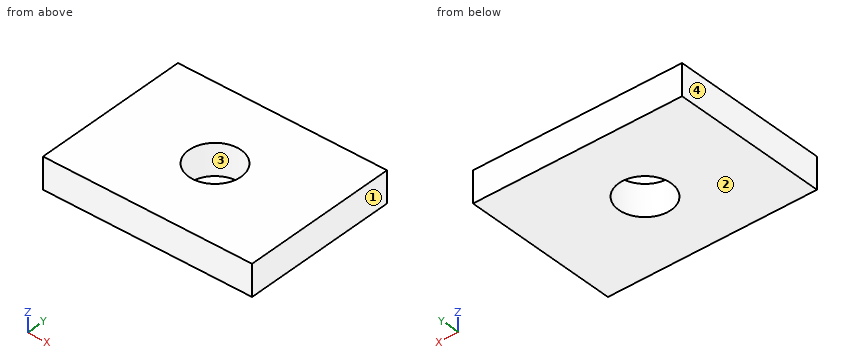
from build123d import *

# Parameters (mm, degrees)
SKETCH1_W           = 40
SKETCH1_H           = 30
BOSS_EXTRUDE1_DEPTH = 6
SKETCH2_R           = 5
CUT_EXTRUDE1_DEPTH  = 6


with BuildPart() as part:
    # Sketch1 → Boss-Extrude1 (new body)
    with BuildSketch(Plane.XY):
        with Locations((-26.669019685, -3.132226563)):
            Rectangle(SKETCH1_W, SKETCH1_H)
    extrude(amount=BOSS_EXTRUDE1_DEPTH)

    # Sketch2 → Cut-Extrude1 (cut)
    with BuildSketch(Plane.XY.offset(6)):
        with Locations((-26.669019685, -3.132226563)):
            Circle(SKETCH2_R)
    extrude(amount=-CUT_EXTRUDE1_DEPTH, mode=Mode.SUBTRACT)


solid = part.part
Here's how the part is built. I have some questions about the finished solid (model axes, mm). Face numbers are marked on the shaded views. Coordinates: 2 decimals unless noted, no trailing zeros. Order: outer loops, then holes, each group sorted by start corner. A loop starts at its lowest first (then second) coordinate and runs counter-clockwise, first axis right, second up. Notation, with made-up numbers: M 14.5,-31 L 44.5,-31 A23 cw 44.5,-13 Z; hole C 58.5,-6.5 d1. An arc over 180 degrees is marked long. Answer as CSV lines item,"result".
Item 1: Imagine slicing it at B-B on z = 2.1. Write out the boundary of the cut face in (x, y).
Results found:
outline,"M -46.67,-18.13 L -6.67,-18.13 L -6.67,11.87 L -46.67,11.87 Z; hole C -26.67,-3.13 d10"
Item 2: We'd pull the mould along X, two halves only. Please class the marked faces 1, 2, 3 and 4: +X half, -X half, draft (parallel to the pull), parting line (faces both ways), or undercut.
Results found:
face 1,"+X half"
face 2,"draft"
face 3,"undercut"
face 4,"-X half"
Item 3: Imagine slicing it at A-A on y = -7.25. Write out the boundary of the cut face in (x, z).
Results found:
outline,"M -46.67,0 L -29.51,0 L -29.51,6 L -46.67,6 Z; M -23.83,0 L -6.67,0 L -6.67,6 L -23.83,6 Z"
Item 4: If I drill on line 1 (X direction, y = -3, z = 3.1); line 2 (Y direction, x = -24, z = 5.45); line 3 (Y direction, x = -27, z = 3.7), over which ranges is the centre line in solid material (lowest first)?
Results found:
line 1,"-46.67 to -31.67, -21.67 to -6.67"
line 2,"-18.13 to -7.36, 1.1 to 11.87"
line 3,"-18.13 to -8.12, 1.86 to 11.87"
Item 5: Imagine slicing it at C-C on y = -4. Write out the boundary of the cut face in (x, z), plus the area to 3 significant figures.
Results found:
outline,"M -46.67,0 L -31.59,0 L -31.59,6 L -46.67,6 Z; M -21.74,0 L -6.67,0 L -6.67,6 L -21.74,6 Z"
area,"181 mm2"
